Verification items for the finished model (mm, model axes). A direction names the side the tool comes from. Coordinates: 2 decimals unless noted, no trailing zeros. Write each loop counter-clockwise with the first axis right and the second up, starting at its lowest first coordinate (ties: lowest second). Pieces come first, ordered by that corner, then holes. Notation, with made-up numbers: (-1, 73.25) -> (6, 73.25) arc R23 cw to (6, 107.25) -> close; hole circle Ø5 at (43.5, 1.5). An arc over 180 degrees is marked (long way). Use CSV: the item, a comma, the result in double quotes.
```python
from build123d import *

# Parameters (mm, degrees)
BASE_PLATE_DEPTH         = 15
PIVOT_BOSS_1_PROFILE_R   = 24
PIVOT_BOSS_1_DEPTH       = 22
PIVOT_START              = -22
PIVOT_BOSS_2_PROFILE_R   = 24
PIVOT_BOSS_2_DEPTH       = 22
UPRIGHT_WEB_DEPTH        = 15
WEB_SLOT_DEPTH           = 55
WEB_HOLE_PROFILE_R       = 10
WEB_HOLE_DEPTH           = 55
PIVOT_BORE_PROFILE_R     = 9
PIVOT_BORE_THROUGH_DEPTH = 90


with BuildPart() as part:
    # Base Plate Profile → Base Plate (new body)
    with BuildSketch(Plane.XY):
        with BuildLine():
            Line((0, 0), (64, 0))
            Line((64, 0), (64, -22))
            Line((64, -22), (27.24, -22))
            ThreePointArc((27.24, -22), (18.754718626, -25.514718626), (15.24, -34))
            Line((15.24, -34), (15.24, -54))
            ThreePointArc((15.24, -54), (18.754718626, -62.485281374), (27.24, -66))
            Line((27.24, -66), (64, -66))
            Line((64, -66), (64, -88))
            Line((64, -88), (0, -88))
            Line((0, -88), (0, 0))
        make_face()
    extrude(amount=BASE_PLATE_DEPTH)

    # Pivot Boss 1 Profile → Pivot Boss 1 (add)
    with BuildSketch(Plane(origin=(0, 0, 0), x_dir=(1, 0, 0), z_dir=(0, 1, 0))):
        with Locations((64, -24)):
            Circle(PIVOT_BOSS_1_PROFILE_R)
    extrude(amount=-PIVOT_BOSS_1_DEPTH)

    # Pivot Boss 2 Profile → Pivot Boss 2 (add)
    with BuildSketch(Plane.XZ.offset(88).offset(PIVOT_START)):
        with Locations((64, 24)):
            Circle(PIVOT_BOSS_2_PROFILE_R)
    extrude(amount=PIVOT_BOSS_2_DEPTH)

    # Upright Web Profile → Upright Web (add)
    with BuildSketch(Plane(origin=(0, 0, 0), x_dir=(-1, 0, 0), z_dir=(0, 0, -1))):
        with BuildLine():
            Line((0, -44), (0, -17))
            Line((0, -17), (0, -5))
            ThreePointArc((0, -5), (3.514718626, -13.485281374), (12, -17))
            Line((12, -17), (50, -17))
            Line((50, -17), (50, -71))
            Line((50, -71), (12, -71))
            ThreePointArc((12, -71), (3.514718626, -74.514718626), (0, -83))
            Line((0, -83), (0, -71))
            Line((0, -71), (0, -44))
        make_face()
    extrude(amount=-UPRIGHT_WEB_DEPTH)

    # Web Slot Profile → Web Slot (cut)
    with BuildSketch(Plane(origin=(0, -17, 0), x_dir=(1, 0, 0), z_dir=(0, 1, 0))):
        Polygon((-50, -7.5), (-50, -6.5), (-18, -6.5), (-18, -8.5), (-50, -8.5), align=None)
    extrude(amount=-WEB_SLOT_DEPTH, mode=Mode.SUBTRACT)

    # Web Hole Profile → Web Hole (cut)
    with BuildSketch(Plane.XY.offset(15)):
        with Locations((-31, -44)):
            Circle(WEB_HOLE_PROFILE_R)
    extrude(amount=-WEB_HOLE_DEPTH, mode=Mode.SUBTRACT)

    # Pivot Bore Profile → Pivot Bore Through (cut)
    with BuildSketch(Plane(origin=(0, 0, 0), x_dir=(1, 0, 0), z_dir=(0, 1, 0))):
        with Locations(Location((64, -24, 0), (0, 0, 270))):
            Circle(PIVOT_BORE_PROFILE_R)
    extrude(amount=-PIVOT_BORE_THROUGH_DEPTH, mode=Mode.SUBTRACT)


solid = part.part
```
1) Mould release check, pull along Z, two halves, no side actions. Record for faces 5 (the cylindrical face through (-33.17, -53.76, 3.3)), 6 (the flat face through (8, -43, 0)), 7 (the flat face through (-41, -38, 8.5)), 8 (the flat face through (-41.3, -43.6, 6.5)): released by +Z, released by -Z, zero draft, split by the parting line, or undercut.
Return value:
face 5,"zero draft"
face 6,"released by -Z"
face 7,"undercut"
face 8,"undercut"
2) Cross-section at A-A (x = -23). Record the boundary of the cut face in (y, z).
Return value:
outline,"(-71, 0) -> (-50, 0) -> (-50, 6.5) -> (-71, 6.5) -> close; (-71, 8.5) -> (-50, 8.5) -> (-50, 15) -> (-71, 15) -> close; (-38, 0) -> (-17, 0) -> (-17, 6.5) -> (-38, 6.5) -> close; (-38, 8.5) -> (-17, 8.5) -> (-17, 15) -> (-38, 15) -> close"
3) Cross-section at D-D (x = 20). Record the boundary of the cut face in (y, z).
Return value:
outline,"(-88, 0) -> (-63.57, 0) -> (-63.57, 15) -> (-88, 15) -> close; (-24.43, 0) -> (0, 0) -> (0, 15) -> (-24.43, 15) -> close"
4) Gauge pin test, flat ends, axial feed: pin 1 (5.5 mm diameter, centred on y = -85, z = 6.5, fed in from -X); pin 2 (8 mm diameter, centred on x = 63.5, z = 32.5, fed in from +Y); pin 3 (2 mm diameter, centred on y = -76, z = 36, fed in from +X); pin 4 (4 mm diameter, centred on y = -74, z = 30, fed in from -X). Record the tip position at first contact, or that the pin passes through.
Return value:
pin 1,"x = -0.02"
pin 2,"y = 0"
pin 3,"x = 85.33"
pin 4,"x = 40.34"
5) Scan lines: L1, parallel to X at y = -5.25, z = 24; L2, parallel to Y at x = 62.5, z = 36.5; L3, parallel to Z at x = -19, y = -51.5. Record each from-to range of solid material in increasing order.
Return value:
L1,"40 to 55, 73 to 88"
L2,"-88 to -66, -22 to 0"
L3,"0 to 6.5, 8.5 to 15"
6) Cross-section at B-B (y = -18.5). Record the boundary of the cut face in (x, z).
Return value:
outline,"(-50, 0) -> (64, 0) arc R24 ccw (long way) to (41.75, 15) -> (-50, 15) -> (-50, 8.5) -> (-18, 8.5) -> (-18, 6.5) -> (-50, 6.5) -> close; hole circle Ø18 at (64, 24)"
7) Cross-section at C-C (z = 24). Record the boundary of the cut face in (x, y), plus the area to 3 significant figures.
Return value:
outline,"(40, -88) -> (55, -88) -> (55, -66) -> (40, -66) -> close; (40, -22) -> (55, -22) -> (55, 0) -> (40, 0) -> close; (73, -88) -> (88, -88) -> (88, -66) -> (73, -66) -> close; (73, -22) -> (88, -22) -> (88, 0) -> (73, 0) -> close"
area,"1,320 mm2"
8) Set-up check for faces 1 (the flat face through (57, -22, 13)), 2 (the flat face through (-31, -17, 9)), 3 (the flat face through (-50, -44, 12)), 4 (the flat face through (-31, -71, 9)): record each of +Z, -Z, +X, -X, +Y, -Y from which the full face is reachable in a straight line by a thin tool's end or side.
Return value:
face 1,"+Z, -Z, +X"
face 2,"+Z, -Z, -X, +Y"
face 3,"+Z, -Z, -X, +Y, -Y"
face 4,"+Z, -Z, -X, -Y"
